from build123d import *

# Parameters (mm, degrees)
HUB_SKETCH_60_R       = 30
HUB_60X50_DEPTH       = 25
BORE_SKETCH_30_R      = 15
HUB_BORE_30_DEPTH     = 66.574385243
ARM_PLATE_10MM_DEPTH  = 5
CLEVIS_BASE_DEPTH     = 10
CLEVIS_LUG_1_SKETCH_R = 6
CLEVIS_LUG_1_DEPTH    = 9
CLEVIS_START          = -9
CLEVIS_LUG_2_SKETCH_R = 6
CLEVIS_LUG_2_DEPTH    = 9


with BuildPart() as part:
    # Hub Sketch Ø60 → Hub Ø60x50 (new, symmetric)
    with BuildSketch(Plane(origin=(0, 0, 0), x_dir=(1, 0, 0), z_dir=(0, 1, 0))):
        with Locations(Location((0, 0, 0), (0, 0, 270))):
            Circle(HUB_SKETCH_60_R)
    extrude(amount=HUB_60X50_DEPTH, both=True)

    # Bore Sketch Ø30 → Hub Bore Ø30 (cut, through all)
    with BuildSketch(Plane(origin=(0, 25, 0), x_dir=(1, 0, 0), z_dir=(0, 1, 0))):
        with Locations(Location((0, 0, 0), (0, 0, 270))):
            Circle(BORE_SKETCH_30_R)
    extrude(amount=-HUB_BORE_30_DEPTH, mode=Mode.SUBTRACT)

    # Arm Plate Sketch → Arm Plate 10mm (add, symmetric)
    with BuildSketch(Plane(origin=(0, 0, 0), x_dir=(1, 0, 0), z_dir=(0, 1, 0))):
        with BuildLine():
            Line((-101.962487217, 15), (-4.462487217, 29.666246946))
            ThreePointArc((-4.462487217, 29.666246946), (-30, 0), (-4.462487217, -29.666246946))
            Line((-4.462487217, -29.666246946), (-101.962487217, -15))
            Line((-101.962487217, -15), (-101.962487217, 15))
        make_face()
    extrude(amount=ARM_PLATE_10MM_DEPTH, both=True)

    # Clevis Base Sketch → Clevis Base (add)
    with BuildSketch(Plane(origin=(0, 5, 0), x_dir=(1, 0, 0), z_dir=(0, 1, 0))):
        with BuildLine():
            Line((-101.962487217, -15), (-126.962487217, -15))
            Line((-126.962487217, -15), (-126.962487217, 15))
            Line((-126.962487217, 15), (-101.962487217, 15))
            Line((-101.962487217, 15), (-4.462487217, 29.666246946))
            ThreePointArc((-4.462487217, 29.666246946), (-30, 0), (-4.462487217, -29.666246946))
            Line((-4.462487217, -29.666246946), (-101.962487217, -15))
        make_face()
    extrude(amount=-CLEVIS_BASE_DEPTH)

    # Clevis Lug 1 Sketch → Clevis Lug 1 (add)
    with BuildSketch(Plane.XY.offset(15)):
        with BuildLine():
            Line((-101.962487217, 5), (-101.962487217, 20.272052395))
            ThreePointArc((-101.962487217, 20.272052395), (-114.462487217, 32.772052395), (-126.962487217, 20.272052395))
            Line((-126.962487217, 20.272052395), (-126.962487217, 5))
            Line((-126.962487217, 5), (-101.962487217, 5))
        make_face()
        with Locations((-114.462487217, 20.272052395)):
            Circle(CLEVIS_LUG_1_SKETCH_R, mode=Mode.SUBTRACT)
    extrude(amount=-CLEVIS_LUG_1_DEPTH)

    # Clevis Lug 2 Sketch → Clevis Lug 2 (add)
    with BuildSketch(Plane(origin=(0, 0, -15), x_dir=(-1, 0, 0), z_dir=(0, 0, -1)).offset(CLEVIS_START)):
        with BuildLine():
            Line((126.962487217, 20.272052395), (126.962487217, 5))
            Line((126.962487217, 5), (101.962487217, 5))
            Line((101.962487217, 5), (101.962487217, 20.272052395))
            ThreePointArc((101.962487217, 20.272052395), (114.462487217, 32.772052395), (126.962487217, 20.272052395))
        make_face()
        with Locations(Location((114.462487217, 20.272052395, 0), (0, 0, 180))):
            Circle(CLEVIS_LUG_2_SKETCH_R, mode=Mode.SUBTRACT)
    extrude(amount=CLEVIS_LUG_2_DEPTH)


solid = part.part
Work out the finished part from the listing and answer in its coordinate system (mm). A direction names the side the tool comes from. Round coordinates to 2 decimals unless told otherwise and drop trailing zeros. Loops run counter-clockwise (first coordinate to the right, second up) from the corner with the lowest first, then second, coordinate; pieces in that order, holes last. Notation, with made-up numbers: (-0.75, 26) - (45.25, 26) arc R28 ccw to (45.25, 47) - close; hole circle Ø4 at (12, -37.5). An arc over 180 degrees is marked (long way). One line per item, written item: value.
Q1. Find section D-D on y = 16. Give the vertices of the cut face in (x, z).
Check values:
outline: (-126.96, -15) - (-118.68, -15) - (-118.68, -6) - (-126.96, -6) - close; (-126.96, 6) - (-118.68, 6) - (-118.68, 15) - (-126.96, 15) - close; (-110.25, -15) - (-101.96, -15) - (-101.96, -6) - (-110.25, -6) - close; (-110.25, 6) - (-101.96, 6) - (-101.96, 15) - (-110.25, 15) - close; circle Ø60 at (0, 0); hole circle Ø30 at (0, 0)
Q2. The mould has two halves that part along X. Classify faces 1 (the flat face through (-52.53, 0.07, 22.436)), 2 (the flat face through (-65, 5, 0)), 3 (the cylindrical face through (-108.92, 17.97, 10.56)), 4 (the flat face through (-115, 13, -6)): +X half, -X half, draft (parallel to the pull), parting line (faces both ways), or undercut.
Check values:
face 1: -X half
face 2: undercut
face 3: undercut
face 4: draft
Q3. Each of these flat-tipped pins is pushed along its axis until it touches: pin 1 Ø18 at (x, z) = (-88.5, 7.5) entering from -Y; pin 2 Ø4 at (y, z) = (6, 16) entering from +X; pin 3 Ø5 at (y, z) = (14.5, -24) entering from -X. Where does it stop, or does it pass through?
Check values:
pin 1: y = -5
pin 2: x = 26.53
pin 3: x = -20.92
Q4. For faces 5 (the flat face through (-101.962, 13, -10)), 6 (the flat face through (-115, 10, -15)), 7 (the flat face through (-115, 13, 6)), 8 (the flat face through (-115, 10, 15)), 9 (the flat face through (14, 25, 6)), determine the directions among +Z, -Z, +X, -X, +Y, -Y from which every point of the face is accessible in a straight line to the end or side of a thin tool.
Check values:
face 5: +Z, -Z, +Y
face 6: -Z, -X, +Y, -Y
face 7: -X, +Y
face 8: +Z, -X, +Y, -Y
face 9: +Z, -Z, +X, +Y
Q5. Find section C-C on y = 23. Give the vertices of the cut face in (x, z).
Check values:
outline: (-126.66, -15) - (-119.81, -15) - (-119.81, -6) - (-126.66, -6) - close; (-126.66, 6) - (-119.81, 6) - (-119.81, 15) - (-126.66, 15) - close; (-109.12, -15) - (-102.26, -15) - (-102.26, -6) - (-109.12, -6) - close; (-109.12, 6) - (-102.26, 6) - (-102.26, 15) - (-109.12, 15) - close; circle Ø60 at (0, 0); hole circle Ø30 at (0, 0)
Q6. Find section A-A on x = 0. Give the vertices of the cut face in (y, z), and give its area (3 significant figures).
Check values:
outline: (-25, -30) - (25, -30) - (25, -15) - (-25, -15) - close; (-25, 15) - (25, 15) - (25, 30) - (-25, 30) - close
area: 1,500 mm2
Q7. Find section B-B on z = 0. Give the vertices of the cut face in (x, y).
Check values:
outline: (-126.96, -5) - (-30, -5) - (-30, -25) - (-15, -25) - (-15, 25) - (-30, 25) - (-30, 5) - (-126.96, 5) - close; (15, -25) - (30, -25) - (30, 25) - (15, 25) - close
Q8. Straight lines are drawn through the part: probe 1 along X at (y, z) = (1, -1); probe 2 along Z at (x, y) = (-112.5, 6); probe 3 along X at (y, z) = (22, 1). For each, find the intervals that lie inside material, in ascending order.
Check values:
probe 1: -126.96 to -14.97, 14.97 to 29.98
probe 2: -15 to -6, 6 to 15
probe 3: -29.98 to -14.97, 14.97 to 29.98
